```python
from build123d import *

# Parameters (mm, degrees)
SKETCH1_R           = 6.5
BOSS_EXTRUDE1_DEPTH = 6
CHAMFER1_SIZE       = 2
CHAMFER2_SIZE       = 1


with BuildPart() as part:
    # Sketch1 → Boss-Extrude1 (new, symmetric)
    with BuildSketch(Plane.XY):
        Polygon((-23, -14), (-23, 14), (-18, 14), (-18, 36), (0.696152423, 30.990381057), (18, 21), (18, -21), (0.696152423, -30.990381057), (-18, -36), (-18, -14), align=None)
        with Locations(Location((0, 0, 0), (0, 0, 180))):
            Circle(SKETCH1_R, mode=Mode.SUBTRACT)
    extrude(amount=BOSS_EXTRUDE1_DEPTH, both=True)

    # Chamfer1
    chamfer1_edges = [part.edges().sort_by_distance(p)[0] for p in [
        (-8.651923789, -33.495190528, -6),
        (9.348076211, -25.995190528, -6),
        (9.348076211, 25.995190528, 6),
        (9.348076211, 25.995190528, -6),
        (-8.651923789, 33.495190528, -6),
        (9.348076211, -25.995190528, 6),
        (-8.651923789, -33.495190528, 6),
        (-8.651923789, 33.495190528, 6),
    ]]
    chamfer(chamfer1_edges, length=CHAMFER1_SIZE)

    # Chamfer2
    chamfer2_edges = [part.edges().sort_by_distance(p)[0] for p in [
        (6.5, 0, 6),
        (6.5, 0, -6),
    ]]
    chamfer(chamfer2_edges, length=CHAMFER2_SIZE)


solid = part.part
```
Verification items for the finished model (mm, model axes). A direction names the side the tool comes from. Round coordinates to 2 decimals unless told otherwise and drop trailing zeros. Write each loop counter-clockwise with the first axis right and the second up, starting at its lowest first coordinate (ties: lowest second). Pieces come first, ordered by that corner, then holes. Notation, with made-up numbers: (-38.75, 11.5) -> (-2.75, 11.5) arc R20 cw to (-2.75, 26.5) -> close; hole circle Ø3 at (81, 49). An arc over 180 degrees is marked (long way). Write each question's results on one line, items separated by ' | '. Start each with the question number.
1. Cross-section at A-A (y = 0). Enter the section's corners in (x, z), then the cut area to 3 significant figures.
2. Set-up check for faces 4 (the flat face through (-21, 14, 0)), 5 (the flat face through (-7, -7, 6)), 6 (the flat face through (-20, -14, 0)): record each of +Z, -Z, +X, -X, +Y, -Y from which the full face is reachable in a straight line by a thin tool's end or side.
3. Cross-section at C-C (x = -9.5). Enter the section's corners in (y, z).
4. Material ranges on probe 1 along X at (y, z) = (2.5, -0.25); probe 2 along X at (y, z) = (4, -1.75); probe 3 along Y at (x, z) = (0.5, 2.25), recorded low to high. Write a range as from..to.
5. Cross-section at D-D (y = -27.5). Enter the section's corners in (x, z), then the cut area to 3 significant figures.
6. Depth check by flat-ended pin: P1, Ø1.5, axis at y = -24.5, z = -2, coming from the +X side; P2, Ø2.5, axis at x = -21.5, z = -2.5, coming from the +Y side; P3, Ø1.5, axis at x = -7, z = 4, coming from the -Y side. Enter the tip coordinate at first touch or a pass-through.
7. Cross-section at B-B (z = 1.25). Enter the section's corners in (x, y), then the cut area to 3 significant figures.
8. Draft check along X on faces 1 (the cylindrical face through (5.158, 3.955, -0.07)), 2 (the flat face through (-8.8, -32.5, 5)), 3 (the flat face through (-18, 25, 0)). Enter one of: +X half, -X half, draft (parallel to the pull), parting line (faces both ways), or undercut.
Solutions:
1) outline: (-23, -6) -> (-7.5, -6) -> (-6.5, -5) -> (-6.5, 5) -> (-7.5, 6) -> (-23, 6) -> close; (6.5, -5) -> (7.5, -6) -> (18, -6) -> (18, 6) -> (7.5, 6) -> (6.5, 5) -> close | area: 334 mm2
2) face 4: +Z, -Z, -X, +Y | face 5: +Z, +X, -X, +Y, -Y | face 6: +Z, -Z, -X, -Y
3) outline: (-33.72, -4) -> (-31.65, -6) -> (31.65, -6) -> (33.72, -4) -> (33.72, 4) -> (31.65, 6) -> (-31.65, 6) -> (-33.72, 4) -> close
4) probe 1: x = -23..-6, 6..18 | probe 2: x = -23..-5.12, 5.12..18 | probe 3: y = -31.04..-6.48, 6.48..31.04
5) outline: (-18, -6) -> (2.74, -6) -> (6.74, -4) -> (6.74, 4) -> (2.74, 6) -> (-18, 6) -> close | area: 289 mm2
6) P1: stops at x = 13.24 | P2: stops at y = 14 | P3: stops at y = -33.25
7) outline: (-23, -14) -> (-18, -14) -> (-18, -36) -> (0.7, -30.99) -> (18, -21) -> (18, 21) -> (0.7, 30.99) -> (-18, 36) -> (-18, 14) -> (-23, 14) -> close; hole circle Ø13 at (0, 0) | area: 2,160 mm2
8) face 1: undercut | face 2: +X half | face 3: -X half
